Geometry check sheet. Reference: drawing and pictorial views, mm from the part's lowest x, y, z. A direction names the side the tool comes from. Round coordinates to 2 decimals unless told otherwise and drop trailing zeros. Loops run counter-clockwise (first coordinate to the right, second up) from the corner with the lowest first, then second, coordinate; pieces in that order, holes last. Notation, with made-up numbers: (77.25, -15) - (118.25, -15) arc R35 cw to (118.25, 24) - close; hole circle Ø9 at (-17.75, 44.5). An arc over 180 degrees is marked (long way). Return JSON: item names as keys, results as strings.
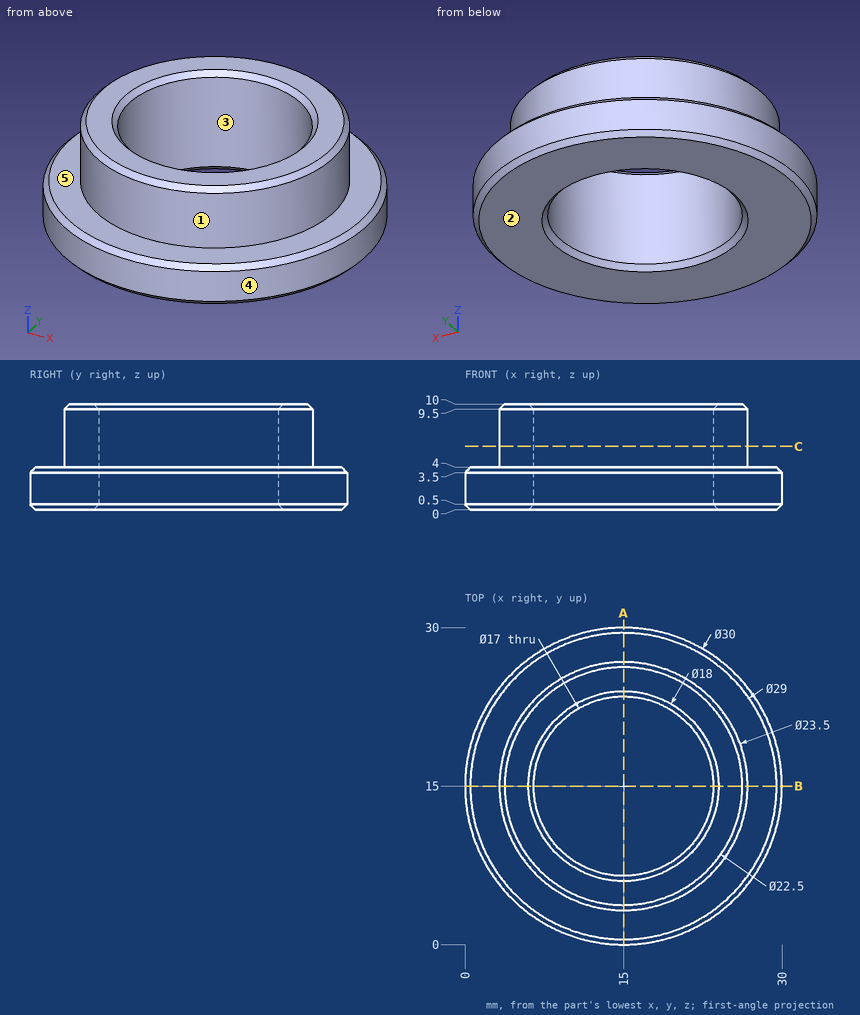
Q1. Scan lines: probe 1 along Y at (x, z) = (15, 6.5); probe 2 along Y at (x, z) = (15, 2.5); probe 3 along X at (y, z) = (12.5, 8.5). Record each from-to range of solid material in increasing order. Write a range as [from, to].
Answer key:
{"probe 1": "y = [3.25, 6.5], [23.5, 26.75]", "probe 2": "y = [0, 6.5], [23.5, 30]", "probe 3": "x = [3.52, 6.88], [23.12, 26.48]"}
Q2. Draft check along X on the marked faces 3, 4 and 5. Enter one of: released by +X, released by -X, zero draft, split by the parting line, or undercut.
Answer key:
{"face 3": "undercut", "face 4": "split by the parting line", "face 5": "zero draft"}
Q3. Sectioned sample at A-A (x = 15). Enter the section's corners in (y, z), plus the area to 4 significant figures.
Answer key:
{"outline": "(0, 0.5) - (0.5, 0) - (6, 0) - (6.5, 0.5) - (6.5, 9.5) - (6, 10) - (3.75, 10) - (3.25, 9.5) - (3.25, 4) - (0.5, 4) - (0, 3.5) - close; (23.5, 0.5) - (24, 0) - (29.5, 0) - (30, 0.5) - (30, 3.5) - (29.5, 4) - (26.75, 4) - (26.75, 9.5) - (26.25, 10) - (24, 10) - (23.5, 9.5) - close", "area": "89.75 mm²"}
Q4. Sectioned sample at C-C (z = 6). Enter the section's corners in (x, y), plus the area to 3 significant figures.
Answer key:
{"outline": "circle Ø23.5 at (15, 15); hole circle Ø17 at (15, 15)", "area": "207 mm²"}
Q5. Depth check by flat-ended pin: P1, Ø1, axis at x = 23, z = 7, coming from the +Y side (3 decimals); P2, Ø4, axis at x = 11.5, z = 5.5, coming from the +Y side; P3, Ø2, axis at x = 6, z = 9, coming from the +Y side. Enter the tip coordinate at first touch or a pass-through.
Answer key:
{"P1": "stops at y = 24.045", "P2": "stops at y = 29.63", "P3": "stops at y = 23.61"}
Q6. Tool access check on the marked faces 1 and 2. Record the directions out of +Z, -Z, +X, -X, +Y, -Y that give a thin tool (end or side, any length) a straight path to the whole face; none if there is none.
Answer key:
{"face 1": "+Z", "face 2": "-Z, +X, -X, +Y, -Y"}
